from build123d import *


with BuildPart() as part:
    # 草图1 → 旋转1 (revolve)
    with BuildSketch(Plane(origin=(0, 0, 0), x_dir=(0, 0, -1), z_dir=(1, 0, 0)), mode=Mode.PRIVATE) as revolve_1_sk:
        Polygon((53.611052376, 10), (69.611052376, 10), (77.111052376, 16), (99.611052376, 16), (99.611052376, 19), (77.111052376, 19), (69.611052376, 12.5), (53.611052376, 12.5), align=None)
    revolve(revolve_1_sk.sketch.rotate(Axis((0, 0, 0), (0, 0, -1)), 90), axis=Axis((0, 0, 0), (0, 0, -1)))


solid = part.part
Geometry: final body of the model. Coordinates: model frame, mm. Round coordinates to 2 decimals unless told otherwise and drop trailing zeros. Loops run counter-clockwise (first coordinate to the right, second up) from the corner with the lowest first, then second, coordinate; pieces in that order, holes last. Notation, with made-up numbers: (42.25, 71) -> (89.25, 71) arc R27 ccw to (89.25, 98) -> close; hole circle Ø9 at (-32, -5.75). An arc over 180 degrees is marked (long way). One line per question, with ' | ' between items. Start each with the question number.
1. Section A-A on y = 0. Output: boundary loops of the cut face in (x, z), and give its area (3 significant figures).
2. Mould query, pull axis Y, two halves, no side actions, for faces 1 (the face through (-3.47, 15.62, -88.52)), 2 (the face through (10, 13, -99.611)), 3 (the face through (11.923, -3.755, -61.499)). Classes: pulls with the +Y half, pulls with the -Y half, needs draft (parallel to the pull), parting line crosses it, or undercut.
3. Line query: line 1 along Y through (x, z) = (0, -59); line 2 along Y through (x, z) = (-0.5, -83); line 3 along X through (y, z) = (-10, -95). Output: solid intervals per line, ascending. Write a range as [from, to].
4. Contact query for flat-ended pins moving along their axis: pin 1 (19 mm diameter, centred on x = 0, y = 0, fed in from +Z); pin 2 (8 mm diameter, centred on y = -7, z = -78.5, fed in from -X); pin 3 (5 mm diameter, centred on x = 3.5, z = -62, fed in from -Y); pin 4 (12 mm diameter, centred on x = -12.5, y = 2.5, fed in from +Z). Output: stop coordinate, or through.
5. Section C-C on z = -95.5. Output: boundary loops of the cut face in (x, y), and give its area (3 significant figures).
Returned:
1) outline: (-19, -99.61) -> (-16, -99.61) -> (-16, -77.11) -> (-10, -69.61) -> (-10, -53.61) -> (-12.5, -53.61) -> (-12.5, -69.61) -> (-19, -77.11) -> close; (10, -69.61) -> (16, -77.11) -> (16, -99.61) -> (19, -99.61) -> (19, -77.11) -> (12.5, -69.61) -> (12.5, -53.61) -> (10, -53.61) -> close | area: 256 mm2
2) face 1: undercut | face 2: needs draft | face 3: parting line crosses it
3) line 1: y = [-12.5, -10], [10, 12.5] | line 2: y = [-18.99, -15.99], [15.99, 18.99] | line 3: x = [-16.16, -12.49], [12.49, 16.16]
4) pin 1: passes through | pin 2: stops at x = -18.76 | pin 3: stops at y = -12.46 | pin 4: stops at z = -53.61
5) outline: circle Ø38 at (0, 0); hole circle Ø32 at (0, 0) | area: 330 mm2
